Verification items for the finished model (mm, model axes). A direction names the side the tool comes from. Coordinates: 2 decimals unless noted, no trailing zeros. Order: outer loops, then holes, each group sorted by start corner. A loop starts at its lowest first (then second) coordinate and runs counter-clockwise, first axis right, second up.
Q1. Cross-section at D-D, the plane z = -3. Record the boundary of the cut face in (x, y).
Q2. Thickness scan on line 1 (X direction, y = 2, z = 0); line 2 (X direction, y = 1.9, z = 0.75); line 3 (Z direction, x = 3.5, y = 0.4). Record the ranges inside material, lowest first.
Q3. Cross-section at B-B, the plane y = 0.6. Record the boundary of the cut face in (x, z).
Q4. Depth check by flat-ended pin: P1, Ø1.2, axis at x = 14, y = 3, coming from the -Z side; P2, Ø1, axis at y = 3.5, z = 1, coming from the +X side; P3, Ø2, axis at x = 8, y = 0.5, coming from the +Z side. Enter the tip coordinate at first touch or a pass-through.
Q5. Draft check along X on faces 4 (the flat face through (13, 0, 0)), 5 (the cylindrical face through (-3.5, 2, 0.1)). Enter one of: pulls with the +X half, pulls with the -X half, needs draft (parallel to the pull), parting line crosses it, or undercut.
Q6. Cross-section at C-C, the plane z = 0. Record the boundary of the cut face in (x, y), and give its area (3 significant figures).
Q7. Cross-section at A-A, the plane x = 0. Record the boundary of the cut face in (y, z), and give its area (3 significant figures).
Q8. Set-up check for faces 1 (the cylindrical face through (-2, 2, 0)), 2 (the flat face through (12, 2, -2)), 3 (the flat face through (13, 2, 2)): record each of +Z, -Z, +X, -X, +Y, -Y from which the full face is reachable in a straight line by a thin tool's end or side.
from build123d import *

# Parameters (mm, degrees)
SKETCH1_R           = 4
BOSS_EXTRUDE1_DEPTH = 8
SCALE1_SCALE        = 0.5


with BuildPart() as part:
    # Sketch1 → Boss-Extrude1 (new body)
    with BuildSketch(Plane(origin=(0, 0, 0), x_dir=(1, 0, 0), z_dir=(0, 1, 0))):
        with BuildLine():
            Line((5.744562647, 4), (44.255437353, 4))
            ThreePointArc((44.255437353, 4), (57, 0), (44.255437353, -4))
            Line((44.255437353, -4), (5.744562647, -4))
            ThreePointArc((5.744562647, -4), (-7, 0), (5.744562647, 4))
        make_face()
        with Locations(Location((0, 0, 0), (0, 0, 270))):
            Circle(SKETCH1_R, mode=Mode.SUBTRACT)
        with Locations(Location((50, 0, 0), (0, 0, 270))):
            Circle(SKETCH1_R, mode=Mode.SUBTRACT)
    extrude(amount=BOSS_EXTRUDE1_DEPTH)


with BuildPart() as part_1:
    # Scale1: scaled about (0, 0, 0)
    add(part.part.scale(SCALE1_SCALE))


solid = part_1.part
Check values:
1. outline: (-1.8, 0) - (1.8, 0) - (1.8, 4) - (-1.8, 4) - close; (23.2, 0) - (26.8, 0) - (26.8, 4) - (23.2, 4) - close
2. line 1: x = -3.5 to -2, 2 to 23, 27 to 28.5
2. line 2: x = -3.42 to -1.85, 1.85 to 23.15, 26.85 to 28.42
2. line 3: z = -2 to 2
3. outline: (2.87, -2) - (22.13, -2) arc R3.5 ccw (long way) to (22.13, 2) - (2.87, 2) arc R3.5 ccw (long way) to start; hole circle Ø4 at (0, 0); hole circle Ø4 at (25, 0)
4. P1: stops at z = -2
4. P2: stops at x = 28.46
4. P3: stops at z = 2
5. face 4: needs draft
5. face 5: undercut
6. outline: (-3.5, 0) - (-2, 0) - (-2, 4) - (-3.5, 4) - close; (2, 0) - (23, 0) - (23, 4) - (2, 4) - close; (27, 0) - (28.5, 0) - (28.5, 4) - (27, 4) - close
6. area: 96.0 mm2
7. outline: (0, -3.5) - (4, -3.5) - (4, -2) - (0, -2) - close; (0, 2) - (4, 2) - (4, 3.5) - (0, 3.5) - close
7. area: 12.0 mm2
8. face 1: +Y, -Y
8. face 2: -Z, +Y, -Y
8. face 3: +Z, +Y, -Y
